Check sheet for the modelled part. Datum: model origin and axes. Units: mm. A direction names the side the tool comes from. Round coordinates to 2 decimals unless told otherwise and drop trailing zeros. Loops run counter-clockwise (first coordinate to the right, second up) from the corner with the lowest first, then second, coordinate; pieces in that order, holes last. Notation, with made-up numbers: (1.5, 56.25) -> (7.5, 56.25) arc R11 ccw to (7.5, 73.25) -> close; hole circle Ø8 at (8.5, 45). An arc over 180 degrees is marked (long way). One line per item, written item: value. Start each with the question number.
1. Cross-section at C-C on y = 70. Record the cut outline in (x, z).
2. Cross-section at D-D on z = 31. Record the cut outline in (x, y).
3. Cross-section at B-B on x = 0. Record the cut outline in (y, z), then the cut area to 3 significant figures.
4. Release check for a two-part mould opening along Z. For faces 4 (the face through (-189.86, 59.16, 151.19)), 5 (the face through (-14, -4, 0)), 6 (the face through (-180, 124, 197)) record: +Z half, -Z half, draft (parallel to the pull), parting line (faces both ways), or undercut.
5. Go/stop test with flat-tipped pins: pin 1 (3 mm diameter, centred on x = -145.5, z = 167, fed in from +Y); pin 2 (5 mm diameter, centred on y = -1797, z = 282, fed in from +X); pin 3 (4 mm diameter, centred on y = -810.5, z = 156, fed in from +X). Record where each tip stops, or that it passes through.
6. Set-up check for faces 1 (the face through (47, -30, 108)), 2 (the face through (180, 122, 197)), 3 (the face through (-14, -4, 400)): record each of +Z, -Z, +X, -X, +Y, -Y from which the full face is reachable in a straight line by a thin tool's end or side.
7. Material ranges on L1, parallel to Z at x = 9.5, y = -2430; L2, parallel to Y at x = -90.5, z = 207; L3, parallel to Z at x = -189, y = 70, recorded low to high.
8. Cross-section at A-A on z = 200. Record the cut outline in (x, y).
from build123d import *

# Parameters (mm, degrees)
BOSS_EXTRUDE1_DEPTH     = 400
SKETCH2_R               = 50
CUT_EXTRUDE1_DEPTH      = 400
SKETCH3_R               = 100
BOSS_EXTRUDE2_DEPTH     = 2500
CUT_EXTRUDE2_DEPTH      = 2500
CUT_EXTRUDE2_DEPTH_BACK = 2500
SKETCH4_R               = 50
FILLET1_R               = 10


with BuildPart() as part:
    # Sketch1 → Boss-Extrude1 (new body)
    with BuildSketch(Plane.XY):
        Polygon((-180, 0), (180, 0), (180, 170), (200, 170), (200, -30), (-200, -30), (-200, 170), (-180, 170), align=None)
    extrude(amount=BOSS_EXTRUDE1_DEPTH)

    # Sketch2 → Cut-Extrude1 (cut)
    with BuildSketch(Plane(origin=(200, 0, 0), x_dir=(0, 0, -1), z_dir=(1, 0, 0))):
        with Locations(Location((-200, 70, 0), (0, 0, 90))):
            Circle(SKETCH2_R)
    extrude(amount=-CUT_EXTRUDE1_DEPTH, mode=Mode.SUBTRACT)

    # Sketch3 → Boss-Extrude2 (add)
    with BuildSketch(Plane.XZ.offset(30)):
        with Locations(Location((0, 200, 0), (0, 0, 180))):
            Circle(SKETCH3_R)
    extrude(amount=BOSS_EXTRUDE2_DEPTH)

    # Sketch4 → Cut-Extrude2 (cut, two sides: drawn at the far end of the back side and taken through both)
    with BuildSketch(Plane(origin=(0, 0, 0), x_dir=(0, 0, -1), z_dir=(1, 0, 0)).offset(-CUT_EXTRUDE2_DEPTH_BACK)):
        with Locations(Location((-200, -2430, 0), (0, 0, 180))):
            Circle(SKETCH4_R)
    extrude(amount=CUT_EXTRUDE2_DEPTH + CUT_EXTRUDE2_DEPTH_BACK, mode=Mode.SUBTRACT)

    # Fillet1
    fillet1_edges = [part.edges().sort_by_distance(p)[0] for p in [
        (100, -2530, 200),
    ]]
    fillet(fillet1_edges, radius=FILLET1_R)


solid = part.part
Taken from the geometry:
1. outline: (-200, 0) -> (-180, 0) -> (-180, 150) -> (-200, 150) -> close; (-200, 250) -> (-180, 250) -> (-180, 400) -> (-200, 400) -> close; (180, 0) -> (200, 0) -> (200, 150) -> (180, 150) -> close; (180, 250) -> (200, 250) -> (200, 400) -> (180, 400) -> close
2. outline: (-200, -30) -> (200, -30) -> (200, 170) -> (180, 170) -> (180, 0) -> (-180, 0) -> (-180, 170) -> (-200, 170) -> close
3. outline: (-2530, 110) arc R10 ccw to (-2520, 100) -> (-30, 100) -> (-30, 0) -> (0, 0) -> (0, 400) -> (-30, 400) -> (-30, 300) -> (-2520, 300) arc R10 ccw to (-2530, 290) -> close; hole circle Ø100 at (-2430, 200)
3. area: 504,000 mm2
4. face 4: undercut
4. face 5: -Z half
4. face 6: draft
5. pin 1: stops at y = 0
5. pin 2: stops at x = 60.66
5. pin 3: stops at x = 90.75
6. face 1: -Y
6. face 2: +Z, -Z, +Y
6. face 3: +Z, +X, -X, +Y, -Y
7. L1: z = 100.45 to 150, 250 to 299.55
7. L2: y = -2529.97 to -2479.51, -2380.49 to 0
7. L3: z = 0 to 150, 250 to 400
8. outline: (-200, -30) -> (-100, -30) -> (-100, -2380) -> (100, -2380) -> (100, -30) -> (200, -30) -> (200, 20) -> (180, 20) -> (180, 0) -> (-180, 0) -> (-180, 20) -> (-200, 20) -> close; (-200, 120) -> (-180, 120) -> (-180, 170) -> (-200, 170) -> close; (-100, -2520) arc R10 ccw to (-90, -2530) -> (90, -2530) arc R10 ccw to (100, -2520) -> (100, -2480) -> (-100, -2480) -> close; (180, 120) -> (200, 120) -> (200, 170) -> (180, 170) -> close
